The listing builds one solid part. Answer for the finished solid, in the listing's coordinates (mm). A direction names the side the tool comes from. Coordinates: 2 decimals unless noted, no trailing zeros. Order: outer loops, then holes, each group sorted by start corner. A loop starts at its lowest first (then second) coordinate and runs counter-clockwise, first axis right, second up. Notation, with made-up numbers: (-5.5, 13) -> (0.5, 13) arc R29 cw to (0.5, 50) -> close; hole circle Ø2 at (-24.75, 85.25). An arc over 180 degrees is marked (long way). Return JSON: item names as keys, results as strings.
from build123d import *

# Parameters (mm, degrees)
EXTRUDE_1_DEPTH          = 200
EXTRUDE_1_DEPTH_BACK     = 300
SKETCH_7_R               = 6
CUT_EXTRUDE_2_DEPTH      = 83
CUT_EXTRUDE_3_DEPTH      = 303.063321176
CUT_EXTRUDE_3_DEPTH_BACK = 303.063321176
SKETCH_8_R               = 7
EXTRUDE_START            = 250
EXTRUDE_4_DEPTH          = 250


with BuildPart() as part:
    # Sketch 205 → 凸台-拉伸1 (new, two sides: drawn at the far end of the back side and taken through both)
    with BuildSketch(Plane.XY.offset(-EXTRUDE_1_DEPTH_BACK)):
        with BuildLine():
            Line((-13.5, 15), (13.5, 15))
            ThreePointArc((13.5, 15), (17.035533906, 13.535533906), (18.5, 10))
            Line((18.5, 10), (18.5, -10))
            ThreePointArc((18.5, -10), (17.035533906, -13.535533906), (13.5, -15))
            Line((13.5, -15), (-13.5, -15))
            ThreePointArc((-13.5, -15), (-17.035533906, -13.535533906), (-18.5, -10))
            Line((-18.5, -10), (-18.5, 10))
            ThreePointArc((-18.5, 10), (-17.035533906, 13.535533906), (-13.5, 15))
        make_face()
        with BuildLine():
            Line((-13.5, 12.5), (13.5, 12.5))
            ThreePointArc((13.5, 12.5), (15.267766953, 11.767766953), (16, 10))
            Line((16, 10), (16, -10))
            ThreePointArc((16, -10), (15.267766953, -11.767766953), (13.5, -12.5))
            Line((13.5, -12.5), (-13.5, -12.5))
            ThreePointArc((-13.5, -12.5), (-15.267766953, -11.767766953), (-16, -10))
            Line((-16, -10), (-16, 10))
            ThreePointArc((-16, 10), (-15.267766953, 11.767766953), (-13.5, 12.5))
        make_face(mode=Mode.SUBTRACT)
    extrude(amount=EXTRUDE_1_DEPTH + EXTRUDE_1_DEPTH_BACK)

    # 草图7 → 切除-拉伸2 (cut)
    with BuildSketch(Plane(origin=(0, 15, 0), x_dir=(1, 0, 0), z_dir=(0, 1, 0))):
        with Locations((0, -2)):
            Circle(SKETCH_7_R)
    extrude(amount=-CUT_EXTRUDE_2_DEPTH, mode=Mode.SUBTRACT)

    # 草图8 → 切除-拉伸3 (cut, two sides: drawn at the far end of the back side and taken through both)
    with BuildSketch(Plane(origin=(0, 15, 0), x_dir=(1, 0, 0), z_dir=(0, 1, 0)).offset(-CUT_EXTRUDE_3_DEPTH_BACK)):
        with Locations(Location((0, 260, 0), (0, 0, 180))):
            Circle(SKETCH_8_R)
    extrude(amount=CUT_EXTRUDE_3_DEPTH + CUT_EXTRUDE_3_DEPTH_BACK, mode=Mode.SUBTRACT)

    # 草图11 → 凸台-拉伸4 (add)
    with BuildSketch(Plane(origin=(0, 0, -300), x_dir=(-1, 0, 0), z_dir=(0, 0, -1)).offset(EXTRUDE_START)):
        with BuildLine():
            Line((18.5, -10), (18.5, 10))
            ThreePointArc((18.5, 10), (17.035533906, 13.535533906), (13.5, 15))
            Line((13.5, 15), (-13.5, 15))
            ThreePointArc((-13.5, 15), (-17.035533906, 13.535533906), (-18.5, 10))
            Line((-18.5, 10), (-18.5, -10))
            ThreePointArc((-18.5, -10), (-17.035533906, -13.535533906), (-13.5, -15))
            Line((-13.5, -15), (13.5, -15))
            ThreePointArc((13.5, -15), (17.035533906, -13.535533906), (18.5, -10))
        make_face()
        with BuildLine():
            Line((-16, -12.5), (13.5, -12.5))
            ThreePointArc((13.5, -12.5), (15.267766953, -11.767766953), (16, -10))
            Line((16, -10), (16, 10))
            ThreePointArc((16, 10), (15.267766953, 11.767766953), (13.5, 12.5))
            Line((13.5, 12.5), (-13.5, 12.5))
            ThreePointArc((-13.5, 12.5), (-15.267766953, 11.767766953), (-16, 10))
            Line((-16, 10), (-16, -12.5))
        make_face(mode=Mode.SUBTRACT)
    extrude(amount=-EXTRUDE_4_DEPTH)


solid = part.part
1. The part is cut by section C-C on x = 0. Give the vertices of the cut face in (y, z), and give its area (3 significant figures).
Answer block:
{"outline": "(-15, -550) -> (-12.5, -550) -> (-12.5, -267) -> (-15, -267) -> close; (-15, -253) -> (-12.5, -253) -> (-12.5, -4) -> (-15, -4) -> close; (-15, 8) -> (-12.5, 8) -> (-12.5, 200) -> (-15, 200) -> close; (12.5, -550) -> (15, -550) -> (15, -267) -> (12.5, -267) -> close; (12.5, -253) -> (15, -253) -> (15, -4) -> (12.5, -4) -> close; (12.5, 8) -> (15, 8) -> (15, 200) -> (12.5, 200) -> close", "area": "3,620 mm2"}
2. The part is cut by section B-B on z = -260. Give the vertices of the cut face in (x, y).
Answer block:
{"outline": "(-18.5, -10) arc R5 ccw to (-13.5, -15) -> (-7, -15) -> (-7, -12.5) -> (-13.5, -12.5) arc R2.5 cw to (-16, -10) -> (-16, 10) arc R2.5 cw to (-13.5, 12.5) -> (-7, 12.5) -> (-7, 15) -> (-13.5, 15) arc R5 ccw to (-18.5, 10) -> close; (7, -15) -> (13.5, -15) arc R5 ccw to (18.5, -10) -> (18.5, 10) arc R5 ccw to (13.5, 15) -> (7, 15) -> (7, 12.5) -> (13.5, 12.5) arc R2.5 cw to (16, 10) -> (16, -10) arc R2.5 cw to (13.5, -12.5) -> (7, -12.5) -> close"}
3. This flat-tipped pin is pushed along its axis until it touches: pin 1 Ø11 at (x, z) = (0, -260) entering from +Y. Where does it stop, or does it pass through?
Answer block:
{"pin 1": "passes through"}
4. The part is cut by section A-A on y = -3. Give the vertices of the cut face in (x, z).
Answer block:
{"outline": "(-18.5, -550) -> (-16, -550) -> (-16, 200) -> (-18.5, 200) -> close; (16, -550) -> (18.5, -550) -> (18.5, 200) -> (16, 200) -> close"}
5. Determine the mould class of faces 3 (the face through (-1.301, 13.768, 7.857)), 4 (the face through (18.5, 0, -180)), 5 (the face through (0, -13, -550)) for opening direction Z: pulls with the +Z half, pulls with the -Z half, needs draft (parallel to the pull), parting line crosses it, or undercut.
Answer block:
{"face 3": "undercut", "face 4": "needs draft", "face 5": "pulls with the -Z half"}
6. Consider line 1 (Z direction, x = 0, y = 14.2); line 2 (Y direction, x = 8, z = -137); line 3 (X direction, y = 4.5, z = -36). Determine where each line is inside the solid, lowest interval first. Write a range as from..to.
Answer block:
{"line 1": "z = -550..-267, -253..-4, 8..200", "line 2": "y = -15..-12.5, 12.5..15", "line 3": "x = -18.5..-16, 16..18.5"}
7. For faces 1 (the face through (-16, 0, -180)), 2 (the face through (-18.5, 0, -180)), determine the directions among +Z, -Z, +X, -X, +Y, -Y from which every point of the face is accessible in a straight line to the end or side of a thin tool.
Answer block:
{"face 1": "+Z, -Z", "face 2": "+Z, -Z, -X, +Y, -Y"}
8. The part is cut by section D-D on z = 20. Give the vertices of the cut face in (x, y), and give its area (3 significant figures).
Answer block:
{"outline": "(-18.5, -10) arc R5 ccw to (-13.5, -15) -> (13.5, -15) arc R5 ccw to (18.5, -10) -> (18.5, 10) arc R5 ccw to (13.5, 15) -> (-13.5, 15) arc R5 ccw to (-18.5, 10) -> close; hole (-16, -10) arc R2.5 ccw to (-13.5, -12.5) -> (13.5, -12.5) arc R2.5 ccw to (16, -10) -> (16, 10) arc R2.5 ccw to (13.5, 12.5) -> (-13.5, 12.5) arc R2.5 ccw to (-16, 10) -> close", "area": "294 mm2"}
